The drawing under review shows one solid part. Ordinate dimensions are in mm from its lowest x, y, z. Coordinates: 2 decimals unless noted, no trailing zeros. Write each loop counter-clockwise with the first axis right and the second up, starting at its lowest first coordinate (ties: lowest second). Pieces come first, ordered by that corner, then holes.
1) To check wall thickness, follow line 1 along Y through (x, z) = (5.25, 13.25); line 2 along X through (y, z) = (25.5, 8.25); line 3 along X through (y, z) = (31.5, 13.25) (1 decimal). State the ranges of each line that lie inside material, in increasing order.
2) Insertion check: P1, Ø4, axis at y = 18.5, z = 7.5, coming from the -X side; P2, Ø6, axis at y = 29.5, z = 3.5, coming from the -X side (1 decimal); P3, Ø8, axis at x = 16.5, z = 10, coming from the -Y side. Each pin has a flat end and moves straight along its axis. Give the tip position at first contact, or say it passes through.
3) Mouldability with a two-part tool opening along Z and no side actions: class the marked faces 1, 2, 3 and 4 as pulls with the +Z half, pulls with the -Z half, needs draft (parallel to the pull), parting line crosses it, or undercut.
4) We need section A-A on y = 7.5. Write out the cut boundary in (x, z).
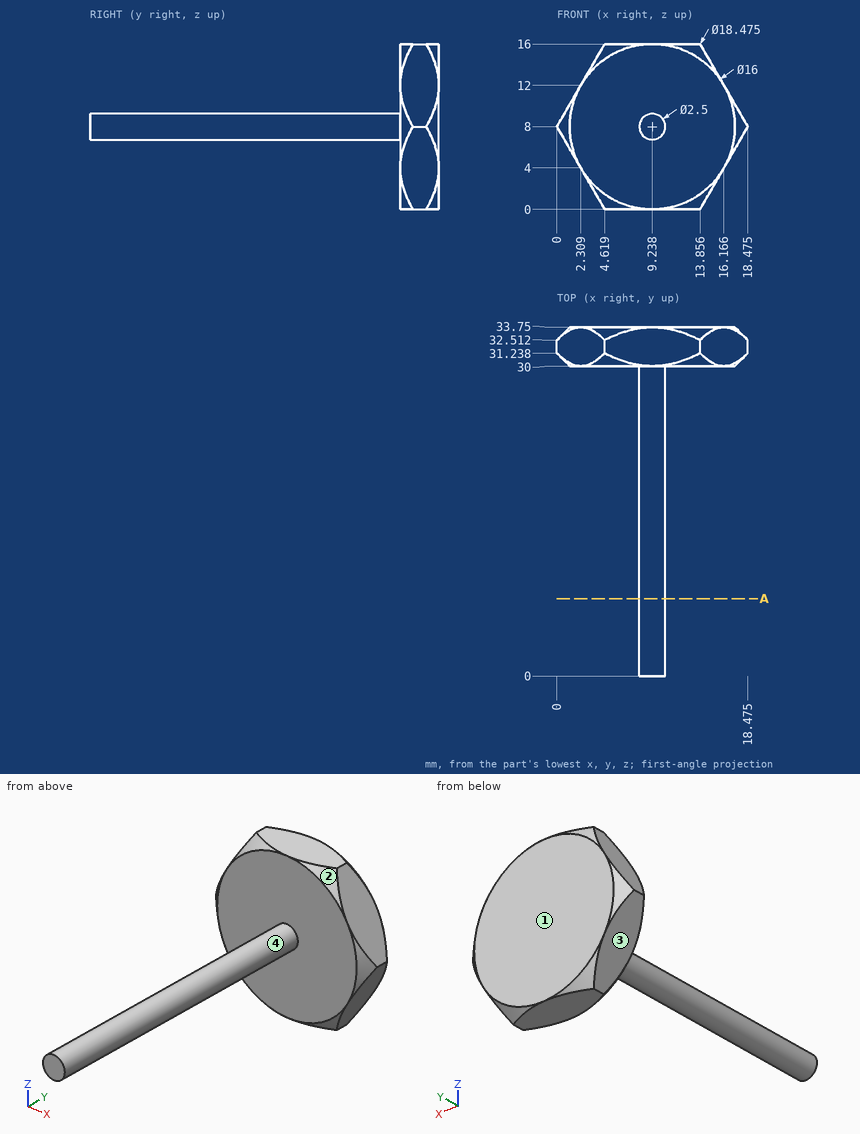
Result:
1. line 1: y = 30 to 33.75
1. line 2: x = 8.01 to 10.46
1. line 3: x = 3 to 15.4
2. P1: stops at x = 7.99
2. P2: stops at x = 1
2. P3: stops at y = 30
3. face 1: needs draft
3. face 2: pulls with the +Z half
3. face 3: pulls with the -Z half
3. face 4: parting line crosses it
4. outline: circle Ø2.5 at (9.24, 8)
